```python
from build123d import *

# Parameters (mm, degrees)
SKETCH1_W          = 55
SKETCH1_H          = 55
BASE_EXTRUDE_DEPTH = 19
SKETCH4_OUTSIDE_W  = 262.948
SKETCH4_OUTSIDE_H  = 262.948
SKETCH4_OUTSIDE_R  = 27.5
CUT_EXTRUDE1_DEPTH = 44.283946216
CUT_EXTRUDE1_DRAFT = -65
FILLET1_R          = 1


with BuildPart() as part:
    # Sketch1 → Base-Extrude (new body)
    with BuildSketch(Plane.XY):
        Rectangle(SKETCH1_W, SKETCH1_H)
    extrude(amount=BASE_EXTRUDE_DEPTH)


with BuildPart() as cut_extrude1_tool:
    # Sketch4 outside → Cut-Extrude1 (with draft: the straight prism first)
    with BuildSketch(Plane.XY.offset(19)):
        Rectangle(SKETCH4_OUTSIDE_W, SKETCH4_OUTSIDE_H)
        Circle(SKETCH4_OUTSIDE_R, mode=Mode.SUBTRACT)
    extrude(amount=-CUT_EXTRUDE1_DEPTH)
    # Cut-Extrude1: the draft: its side faces are tilted about the plane it starts from
    cut_extrude1_sides = [cut_extrude1_tool.faces().sort_by_distance(p)[0] for p in [
        (0, -131.474, -3.141973108),
        (131.474, 0, -3.141973108),
        (0, 131.474, -3.141973108),
        (-131.474, 0, -3.141973108),
        (-27.5, 0, -3.141973108),
    ]]
    draft(cut_extrude1_sides, Plane.XY.offset(19), CUT_EXTRUDE1_DRAFT)


with BuildPart() as part_1:
    add(part.part)

    # Cut-Extrude1: cut by cut_extrude1_tool
    add(cut_extrude1_tool.part, mode=Mode.SUBTRACT)

    # Sketch2 → Boss-Revolve1 (revolve)
    with BuildSketch(Plane(origin=(0, 0, 0), x_dir=(1, 0, 0), z_dir=(0, 1, 0)), mode=Mode.PRIVATE) as boss_revolve1_sk:
        Polygon((0, 0), (13.5, 0), (13.5, 502.401923789), (15, 505), (15, 590), (0, 590), align=None)
    revolve(boss_revolve1_sk.sketch.rotate(Axis((0, 0, -590), (0, 0, 1)), 180), axis=Axis((0, 0, -590), (0, 0, 1)))

    # Fillet1
    fillet1_edges = [part_1.edges().sort_by_distance(p)[0] for p in [
        (13.5, 0, 0),
    ]]
    fillet(fillet1_edges, radius=FILLET1_R)

    # Sketch3 → Cut-Revolve1 (revolve, cut)
    with BuildSketch(Plane(origin=(0, 0, 0), x_dir=(1, 0, 0), z_dir=(0, 1, 0))):
        Polygon((11.969, 590), (15, 591.749948666), (15, 588.250051334), align=None)
    revolve(axis=Axis((0, 0, 0), (0, 0, -1)), mode=Mode.SUBTRACT)


solid = part_1.part
```
Could you check a few things on this model? Use its own coordinates, in mm. A direction names the side the tool comes from. Round coordinates to 2 decimals unless told otherwise and drop trailing zeros. Write each loop counter-clockwise with the first axis right and the second up, starting at its lowest first coordinate (ties: lowest second). Pieces come first, ordered by that corner, then holes. Notation, with made-up numbers: M 26.25,2.25 L 66.25,2.25 A26 ccw 66.25,41.25 Z; hole C 27.5,36.25 d10. An arc over 180 degrees is marked long. Answer in a Markdown table with one row per item. Add a question column.
Q1. Imagine slicing it at A-A (z = -461). Please give me the cut outline in (x, y).
Q2. If I drill on line 1 (Z direction, x = 21, y = 16); line 2 (Y direction, x = -1.5, z = -248), over which ranges is the centre line in solid material (lowest first)? Write a range as from..to.
Q3. Will these pins go through, and if not, where does the flat tip stop? pin 1 Ø4 at (x, y) = (-4.5, -15) entering from -Z; pin 2 Ø12 at (y, z) = (-18, -228.5) entering from +X; pin 3 Ø10 at (y, z) = (10, -378) entering from +X.
Q4. If we mould it in two halves opening along Z, with no side actions, what happens to faces 4 (the flat face through (0, 0, 19)), 5 (the flat face through (-27.5, 0, 9)), 6 (the cylindrical face through (2.93, 13.18, -255.21)), 7 (the flat face through (0, 0, -590))? For each: +Z half, -Z half, draft (parallel to the pull), parting line (faces both ways), or undercut.
Q5. On a 3-axis mill with a long thin cutter (end or side, diameter ignored), from which of +Z, -Z, +X, -X, +Y, -Y can I reach the whole of each face in a straight line? I mean faces 1 (the conical face through (2.9, 13.3, -502.6)), 2 (the cylindrical face through (-8.06, -12.65, -547.21)), 3 (the conical face through (21.287, -21.444, 17.734)). Say none if no direction works.
Values:
| question | item | result |
|---|---|---|
| 1 | outline | C 0,0 d27 |
| 2 | line 1 | 0..19 |
| 2 | line 2 | -13.42..13.42 |
| 3 | pin 1 | z = -589.02 |
| 3 | pin 2 | x = 6.18 |
| 3 | pin 3 | x = 12.54 |
| 4 | face 4 | +Z half |
| 4 | face 5 | draft |
| 4 | face 6 | undercut |
| 4 | face 7 | -Z half |
| 5 | face 1 | none |
| 5 | face 2 | -Z |
| 5 | face 3 | +Z, +X, -Y |
